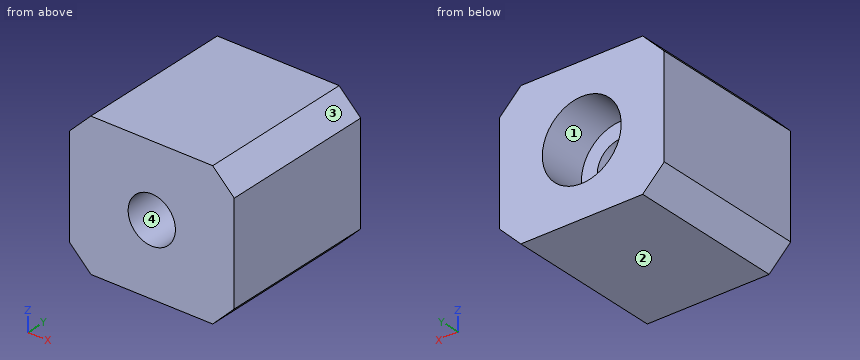
```python
from build123d import *

# Parameters (mm, degrees)
SKETCH_1_W                = 23
SKETCH_1_H                = 22
EXTRUDE_1_DEPTH           = 20
HOLE_WIZARD_1_D           = 6.6
HOLE_WIZARD_1_CBORE_D     = 11
HOLE_WIZARD_1_CBORE_DEPTH = 6.8
CHAMFER_1_SIZE            = 3


with BuildPart() as part:
    # 草图1 → 凸台-拉伸1 (new body)
    with BuildSketch(Plane.XY):
        with Locations((0, 11)):
            Rectangle(SKETCH_1_W, SKETCH_1_H)
    extrude(amount=EXTRUDE_1_DEPTH)

    # 打孔尺寸(%根据)内六角圆柱头螺钉的类型1 (through all)
    with Locations(Plane(origin=(0, 22, 0), x_dir=(1, 0, 0), z_dir=(0, 1, 0))):
        with Locations((0, -10)):
            CounterBoreHole(HOLE_WIZARD_1_D / 2, HOLE_WIZARD_1_CBORE_D / 2, HOLE_WIZARD_1_CBORE_DEPTH)

    # 倒角1
    chamfer_1_edges = [part.edges().sort_by_distance(p)[0] for p in [
        (11.5, 11, 20),
        (-11.5, 11, 20),
        (11.5, 11, 0),
        (-11.5, 11, 0),
    ]]
    chamfer(chamfer_1_edges, length=CHAMFER_1_SIZE)


solid = part.part
```
Build history of the part. All positions in model axes, mm. Face numbers are marked on the shaded views. Coordinates: 2 decimals unless noted, no trailing zeros. Order: outer loops, then holes, each group sorted by start corner. A loop starts at its lowest first (then second) coordinate and runs counter-clockwise, first axis right, second up. Notation, with made-up numbers: (8, 80) -> (63, 80) arc R32 cw to (63, 116) -> close; hole circle Ø6 at (-5, -34.5). An arc over 180 degrees is marked (long way). Answer in a Markdown table with one row per item. Add a question column.
Q1. Band-saw the part on C-C, the plane y = 18.5. List the corners of the cut face in (x, z).
Q2. Band-saw the part on A-A, the plane z = 10. List the corners of the cut face in (x, y), then the cut area to 3 significant figures.
Q3. Band-saw the part on B-B, the plane x = 0. List the corners of the cut face in (y, z), then the cut area to 3 significant figures.
Q4. Wall check: line 1 along Z through (x, y) = (0, 19.5); line 2 along Z through (x, y) = (0, 11); line 3 along X through (y, z) = (9.5, 10). Give the ranges that are in metal, low to high. Write a range as [from, to].
Q5. Band-saw the part on D-D, the plane x = -9.75. List the corners of the cut face in (y, z), then the cut area to 3 significant figures.
Q6. Mould opens along X. For the marked faces 1, 2, 3 and 4 say: +X half, -X half, draft (parallel to the pull), parting line (faces both ways), or undercut.
Q7. Drop a flat-ended pin along its axis: pin 1 (2 mm diameter, centred on x = 2.5, z = 12.5, fed in from +Y). Give the stop position or say it passes through.
Answers follow:
| question | item | result |
|---|---|---|
| 1 | outline | (-11.5, 3) -> (-8.5, 0) -> (8.5, 0) -> (11.5, 3) -> (11.5, 17) -> (8.5, 20) -> (-8.5, 20) -> (-11.5, 17) -> close; hole circle Ø11 at (0, 10) |
| 2 | outline | (-11.5, 0) -> (-3.3, 0) -> (-3.3, 15.2) -> (-5.5, 15.2) -> (-5.5, 22) -> (-11.5, 22) -> close; (3.3, 0) -> (11.5, 0) -> (11.5, 22) -> (5.5, 22) -> (5.5, 15.2) -> (3.3, 15.2) -> close |
| 2 | area | 331 mm^2 |
| 3 | outline | (0, 0) -> (22, 0) -> (22, 4.5) -> (15.2, 4.5) -> (15.2, 6.7) -> (0, 6.7) -> close; (0, 13.3) -> (15.2, 13.3) -> (15.2, 15.5) -> (22, 15.5) -> (22, 20) -> (0, 20) -> close |
| 3 | area | 265 mm^2 |
| 4 | line 1 | [0, 4.5], [15.5, 20] |
| 4 | line 2 | [0, 6.7], [13.3, 20] |
| 4 | line 3 | [-11.5, -3.3], [3.3, 11.5] |
| 5 | outline | (0, 1.25) -> (22, 1.25) -> (22, 18.75) -> (0, 18.75) -> close |
| 5 | area | 385 mm^2 |
| 6 | face 1 | undercut |
| 6 | face 2 | draft |
| 6 | face 3 | +X half |
| 6 | face 4 | undercut |
| 7 | pin 1 | y = 15.2 |
